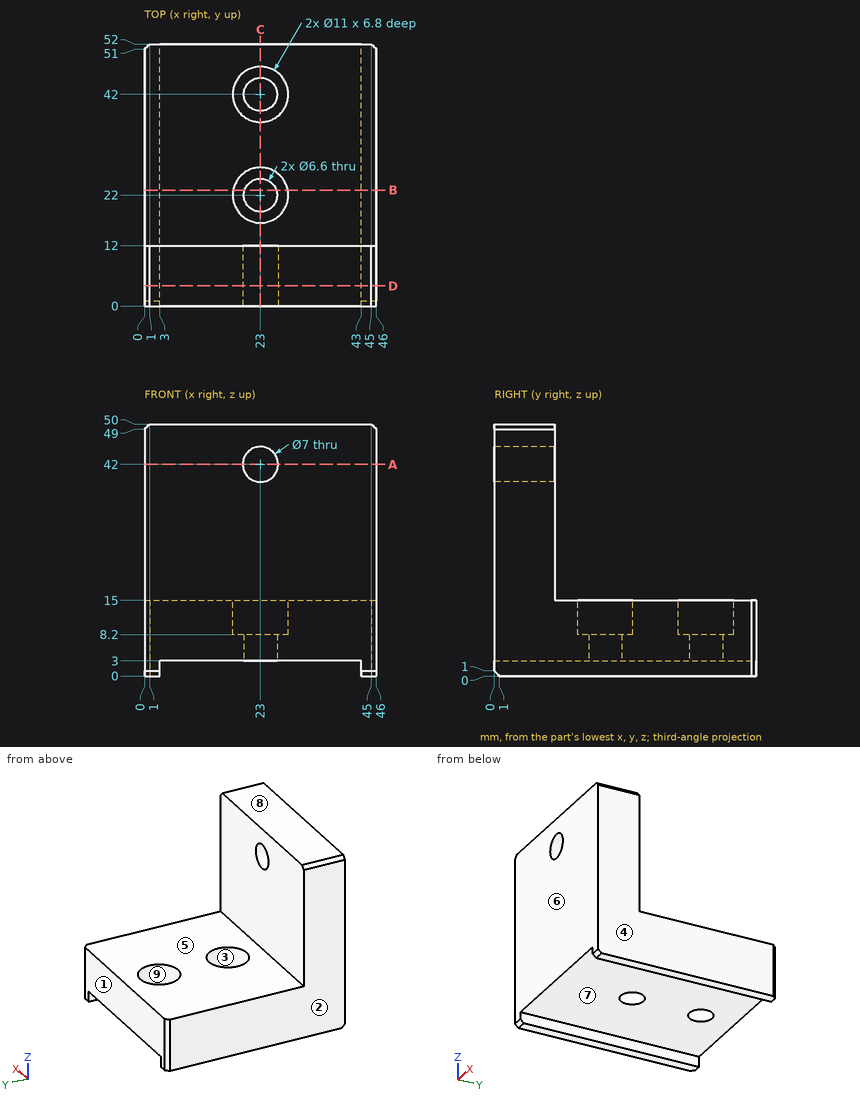
Could you check a few things on this drawing? It's one solid part, dimensions in mm from its lowest x, y, z. A direction names the side the tool comes from. Coordinates: 2 decimals unless noted, no trailing zeros. Loops run counter-clockwise (first coordinate to the right, second up) from the corner with the lowest first, then second, coordinate; pieces in that order, holes last. Notation, with made-up numbers: (25, 14.25) - (82, 14.25) arc R37 ccw to (82, 53.25) - close; hole circle Ø3 at (88, 35). An arc over 180 degrees is marked (long way). Return JSON: item names as keys, results as strings. Group by question number.
Item 1: If we section it at A-A on z = 42: Write out the boundary of the cut face in (x, y).
Item 2: If we section it at D-D on y = 4: Write out the boundary of the cut face in (x, z).
Item 3: I need wall thicknesses on line 1 (Y direction, x = 23, z = 10); line 2 (Y direction, x = 23, z = 6); line 3 (Z direction, x = 44, y = 24). Which ranges of each line are inside material? Lowest first, please. Write a range as from..to.
Item 4: If we section it at B-B on y = 23: Write out the boundary of the cut face in (x, z), and give its area (3 significant figures).
Item 5: If we section it at C-C on x = 23: Write out the boundary of the cut face in (y, z).
Item 6: On a 3-axis mill with a long thin cutter (end or side, diameter ignored), from which of +Z, -Z, +X, -X, +Y, -Y can I reach the whole of each face in a straight line? I mean the marked faces 5, 6, 7, 8 and 9. Say none if no direction works.
Item 7: We'd pull the mould along X, two halves only. Please class the marked faces 1, 2, 3 and 4: +X half, -X half, draft (parallel to the pull), parting line (faces both ways), or undercut.
Item 8: Will these pins go through, and if not, where does the flat tip stop? P1, Ø12, axis at x = 12.5, y = 25, coming from the -Z side; P2, Ø5, axis at x = 29, z = 23.5, coming from the +Y side; P3, Ø4, axis at x = 23, y = 42, coming from the -Z side; P4, Ø6, axis at x = 36.5, y = 37.5, coming from the +Z side.
Calculated:
{
 "1": {"outline": "(0, 0) - (19.5, 0) - (19.5, 12) - (0, 12) - close; (26.5, 0) - (46, 0) - (46, 12) - (26.5, 12) - close"},
 "2": {"outline": "(0, 0) - (3, 0) - (3, 3) - (43, 3) - (43, 0) - (46, 0) - (46, 49) - (45, 50) - (1, 50) - (0, 49) - close; hole circle Ø7 at (23, 42)"},
 "3": {"line 1": "y = 0..16.5, 27.5..36.5, 47.5..52", "line 2": "y = 0..18.7, 25.3..38.7, 45.3..52", "line 3": "z = 0..15"},
 "4": {"outline": "(0, 0) - (3, 0) - (3, 3) - (19.86, 3) - (19.86, 8.2) - (17.59, 8.2) - (17.59, 15) - (0, 15) - close; (26.14, 3) - (43, 3) - (43, 0) - (46, 0) - (46, 15) - (28.41, 15) - (28.41, 8.2) - (26.14, 8.2) - close", "area": "464 mm^2"},
 "5": {"outline": "(0, 3) - (18.7, 3) - (18.7, 8.2) - (16.5, 8.2) - (16.5, 15) - (12, 15) - (12, 38.5) - (0, 38.5) - close; (0, 45.5) - (12, 45.5) - (12, 50) - (0, 50) - close; (25.3, 3) - (38.7, 3) - (38.7, 8.2) - (36.5, 8.2) - (36.5, 15) - (27.5, 15) - (27.5, 8.2) - (25.3, 8.2) - close; (45.3, 3) - (52, 3) - (52, 15) - (47.5, 15) - (47.5, 8.2) - (45.3, 8.2) - close"},
 "6": {"face 5": "+Z, +X, -X, +Y", "face 6": "+Z, -Z, +X, -X, -Y", "face 7": "-Z, +Y, -Y", "face 8": "+Z, +X, -X, +Y, -Y", "face 9": "+Z"},
 "7": {"face 1": "draft", "face 2": "-X half", "face 3": "undercut", "face 4": "+X half"},
 "8": {"P1": "stops at z = 3", "P2": "stops at y = 12", "P3": "passes through", "P4": "stops at z = 15"}
}
